Could you check a few things on this model? Use its own coordinates, in mm. A direction names the side the tool comes from. Give positions to 0.01 mm unless a question says otherwise; leave off trailing zeros. Loops run counter-clockwise (first coordinate to the right, second up) from the corner with the lowest first, then second, coordinate; pieces in that order, holes last. Notation, with made-up numbers: (14, 51) - (55, 51) arc R20 ccw to (55, 66) - close; hole circle Ø6 at (-32, -31.75). An arc over 180 degrees is marked (long way). Write each question's results on one line, items separated by ' | '. Start each with the question number.
```python
from build123d import *

# Parameters (mm, degrees)
CLEVIS_BLOCK_DEPTH         = 22.5
FORK_SLOT_DEPTH            = 64
SIDE_HOLE_A_PROFILE_R      = 12
SIDE_HOLE_A_DEPTH          = 9
SIDE_START                 = -9
SIDE_HOLE_B_PROFILE_R      = 12
SIDE_HOLE_B_DEPTH          = 9
CROSS_HOLE_PROFILE_R       = 6
CROSS_HOLE_DEPTH           = 51
ARM_PLATE_DEPTH            = 4.5
BRACKET_WEB_DEPTH          = 60
PIN_BOSS_PROFILE_R         = 15
PIN_BOSS_DEPTH             = 9
HOOK_SLOT_DEPTH            = 9
BOSS_START                 = -2
BOSS_RECESS_PROFILE_R      = 15
BOSS_RECESS_2MM_DEPTH      = 2
BOSS_START_2               = -16
BOSS_BORE_PROFILE_R        = 15
BOSS_BORE_DEPTH            = 16
BORE_INSERT_BOSS_PROFILE_R = 15
BORE_INSERT_BOSS_DEPTH     = 6.36
INSERT_BORE_PROFILE_R      = 7.5
INSERT_BORE_DEPTH          = 26.36
ARM_TRIM_CUT_DEPTH         = 26.36


with BuildPart() as part:
    # Clevis Block Profile → Clevis Block (new, symmetric)
    with BuildSketch(Plane.XY):
        with BuildLine():
            Line((0, 0), (30, 0))
            Line((30, 0), (30, 60))
            ThreePointArc((30, 60), (0, 90), (-30, 60))
            Line((-30, 60), (-30, 0))
            Line((-30, 0), (0, 0))
        make_face()
    extrude(amount=CLEVIS_BLOCK_DEPTH, both=True)

    # Fork Slot Profile → Fork Slot (cut)
    with BuildSketch(Plane.XY.offset(22.5)):
        with BuildLine():
            Line((0, 0), (9, 0))
            Line((9, 0), (9, 48))
            ThreePointArc((9, 48), (0, 75), (-9, 48))
            Line((-9, 48), (-9, 0))
            Line((-9, 0), (0, 0))
        make_face()
    extrude(amount=-FORK_SLOT_DEPTH, mode=Mode.SUBTRACT)

    # Side Hole A Profile → Side Hole A (cut)
    with BuildSketch(Plane.ZY.offset(30)):
        with Locations((0, 24)):
            Circle(SIDE_HOLE_A_PROFILE_R)
    extrude(amount=-SIDE_HOLE_A_DEPTH, mode=Mode.SUBTRACT)

    # Side Hole B Profile → Side Hole B (cut)
    with BuildSketch(Plane(origin=(30, 0, 0), x_dir=(0, 0, -1), z_dir=(1, 0, 0)).offset(SIDE_START)):
        with Locations(Location((0, 24, 0), (0, 0, 180))):
            Circle(SIDE_HOLE_B_PROFILE_R)
    extrude(amount=SIDE_HOLE_B_DEPTH, mode=Mode.SUBTRACT)

    # Cross Hole Profile → Cross Hole (cut)
    with BuildSketch(Plane(origin=(21, 0, 0), x_dir=(0, 0, -1), z_dir=(1, 0, 0))):
        with Locations(Location((0, 24, 0), (0, 0, 180))):
            Circle(CROSS_HOLE_PROFILE_R)
    extrude(amount=-CROSS_HOLE_DEPTH, mode=Mode.SUBTRACT)

    # Arm Plate Profile → Arm Plate (add, symmetric)
    with BuildSketch(Plane.XY):
        with BuildLine():
            Line((-30, 60), (-30, 150))
            Line((-30, 150), (30, 150))
            Line((30, 150), (30, 60))
            ThreePointArc((30, 60), (0, 90), (-30, 60))
        make_face()
    extrude(amount=ARM_PLATE_DEPTH, both=True)

    # Bracket Web Profile → Bracket Web (add)
    with BuildSketch(Plane(origin=(30, 0, 0), x_dir=(0, 0, -1), z_dir=(1, 0, 0))):
        Polygon((4.5, 150), (-32.976659403, 187.476659403), (-37.476659403, 191.976659403), (-41.976659403, 187.476659403), (-4.5, 150), align=None)
    extrude(amount=-BRACKET_WEB_DEPTH)

    # Pin Boss Profile → Pin Boss (add)
    with BuildSketch(Plane(origin=(0, 72.75, -72.75), x_dir=(1, 0, 0), z_dir=(0, -0.7071067811865479, 0.7071067811865472))):
        with Locations(Location((0, 162.247997693, 0), (0, 0, 270))):
            Circle(PIN_BOSS_PROFILE_R)
    extrude(amount=-PIN_BOSS_DEPTH)

    # Hook Slot Profile → Hook Slot (cut)
    with BuildSketch(Plane(origin=(0, 72.75, -72.75), x_dir=(1, 0, 0), z_dir=(0, -0.7071067811865479, 0.7071067811865472))):
        Polygon((-15, 162.247997693), (-30, 109.247997693), (-30, 162.247997693), align=None)
        Polygon((15, 162.247997693), (30, 109.247997693), (30, 162.247997693), align=None)
    extrude(amount=-HOOK_SLOT_DEPTH, mode=Mode.SUBTRACT)

    # Boss Recess Profile → Boss Recess 2mm (cut)
    with BuildSketch(Plane(origin=(0, 79.113961031, -79.113961031), x_dir=(1, 0, 0), z_dir=(0, 0.7071067811865478, -0.7071067811865472)).offset(BOSS_START)):
        with Locations(Location((0, -162.247997693, 0), (0, 0, 180))):
            Circle(BOSS_RECESS_PROFILE_R)
    extrude(amount=BOSS_RECESS_2MM_DEPTH, mode=Mode.SUBTRACT)

    # Boss Bore Profile → Boss Bore (cut)
    with BuildSketch(Plane(origin=(0, 77.699747468, -77.699747468), x_dir=(1, 0, 0), z_dir=(0, 0.7071067811865479, -0.7071067811865472)).offset(BOSS_START_2)):
        with Locations((0, -162.247997693)):
            Circle(BOSS_BORE_PROFILE_R)
    extrude(amount=BOSS_BORE_DEPTH, mode=Mode.SUBTRACT)

    # Bore Insert Boss Profile → Bore Insert Boss (add)
    with BuildSketch(Plane(origin=(0, 72.75, -72.75), x_dir=(1, 0, 0), z_dir=(0, -0.7071067811865479, 0.7071067811865472))):
        with Locations((0, 162.247997693)):
            Circle(BORE_INSERT_BOSS_PROFILE_R)
    extrude(amount=-BORE_INSERT_BOSS_DEPTH)

    # Insert Bore Profile → Insert Bore (cut)
    with BuildSketch(Plane(origin=(0, 72.75, -72.75), x_dir=(1, 0, 0), z_dir=(0, -0.7071067811865479, 0.7071067811865472))):
        with Locations(Location((0, 162.247997693, 0), (0, 0, 270))):
            Circle(INSERT_BORE_PROFILE_R)
    extrude(amount=-INSERT_BORE_DEPTH, mode=Mode.SUBTRACT)

    # Arm Trim Profile → Arm Trim Cut (cut)
    with BuildSketch(Plane.XY.offset(4.5)):
        with BuildLine():
            Line((0, 111), (30, 111))
            Line((30, 111), (30, 120))
            Line((30, 120), (30, 129))
            Line((30, 129), (0, 129))
            ThreePointArc((0, 129), (-9, 120), (0, 111))
        make_face()
    extrude(amount=-ARM_TRIM_CUT_DEPTH, mode=Mode.SUBTRACT)


solid = part.part
```
Q1. I need wall thicknesses on L1, parallel to Y at x = 23, z = 0; L2, parallel to Z at x = 13, y = 24; L3, parallel to Y at x = 9.5, z = 18.5. Which ranges of each line are inside material? Lowest first, please. Write a range as from..to.
Q2. I want a section at B-B, the plane x = 13. State how many separate pieces and enclosed holes the cut face has, then the cut area to 3 significant figures.
Q3. I want a section at D-D, the plane y = 64.5. List the corners of the cut face in (x, z) for me.
Q4. I want a section at A-A, the plane y = 24. List the corners of the cut face in (x, z) for me, then the cut area to 3 significant figures.
Q5. Which directions (+Z, -Z, +X, -X, +Y, -Y) give clear straight access to the entire face, cutting with the end or side of a thin tool? Please do faces 4 (the face through (-9, 30, 5)), 5 (the face through (25.44, 12.1, -1.56)), 6 (the face through (-0.4, 169, 23.5)).
Q6. I'm going to push flat-ended pins straight in: pin 1 Ø3 at (x, y) = (14, 131.5) entering from -Z; pin 2 Ø2 at (x, z) = (-21, -10.5) entering from -Y; pin 3 Ø21.5 at (y, z) = (24, 0) entering from +X; pin 4 Ø7 at (y, z) = (19, -2) entering from -X. Where does each tip first touch, or does it pass through?
Q7. If we mould it in two halves opening along X, with no side actions, what happens to faces 1 (the face through (0, 106, 4.5)), 2 (the face through (2.253, 184.635, 34.701)), 3 (the face through (-30, 49, 2))? For each: +X half, -X half, draft (parallel to the pull), parting line (faces both ways), or undercut.
Conclusion:
1) L1: 0..12, 36..111, 129..154.5 | L2: -22.5..-6, 6..22.5 | L3: 0..48.39, 71.61..88.46, 164..173
2) separate pieces: 3 | enclosed holes: 1 | area: 3,940 mm^2
3) outline: (-30, -4.5) - (-29.66, -4.5) - (-29.66, -22.5) - (-14.31, -22.5) - (-14.31, 22.5) - (-29.66, 22.5) - (-29.66, 4.5) - (-30, 4.5) - close; (14.31, -22.5) - (29.66, -22.5) - (29.66, -4.5) - (30, -4.5) - (30, 4.5) - (29.66, 4.5) - (29.66, 22.5) - (14.31, 22.5) - close
4) outline: (-30, -22.5) - (-9, -22.5) - (-9, -6) - (-21, -6) - (-21, -12) - (-30, -12) - close; (-30, 12) - (-21, 12) - (-21, 6) - (-9, 6) - (-9, 22.5) - (-30, 22.5) - close; (9, -22.5) - (30, -22.5) - (30, -12) - (21, -12) - (21, -6) - (9, -6) - close; (9, 6) - (21, 6) - (21, 12) - (30, 12) - (30, 22.5) - (9, 22.5) - close | area: 1,170 mm^2
5) face 4: +Z, -Z, -Y | face 5: +X | face 6: +Z, +X, -X
6) pin 1: z = -4.5 | pin 2: y = 0 | pin 3: x = 21 | pin 4: x = -21
7) face 1: draft | face 2: undercut | face 3: -X half
